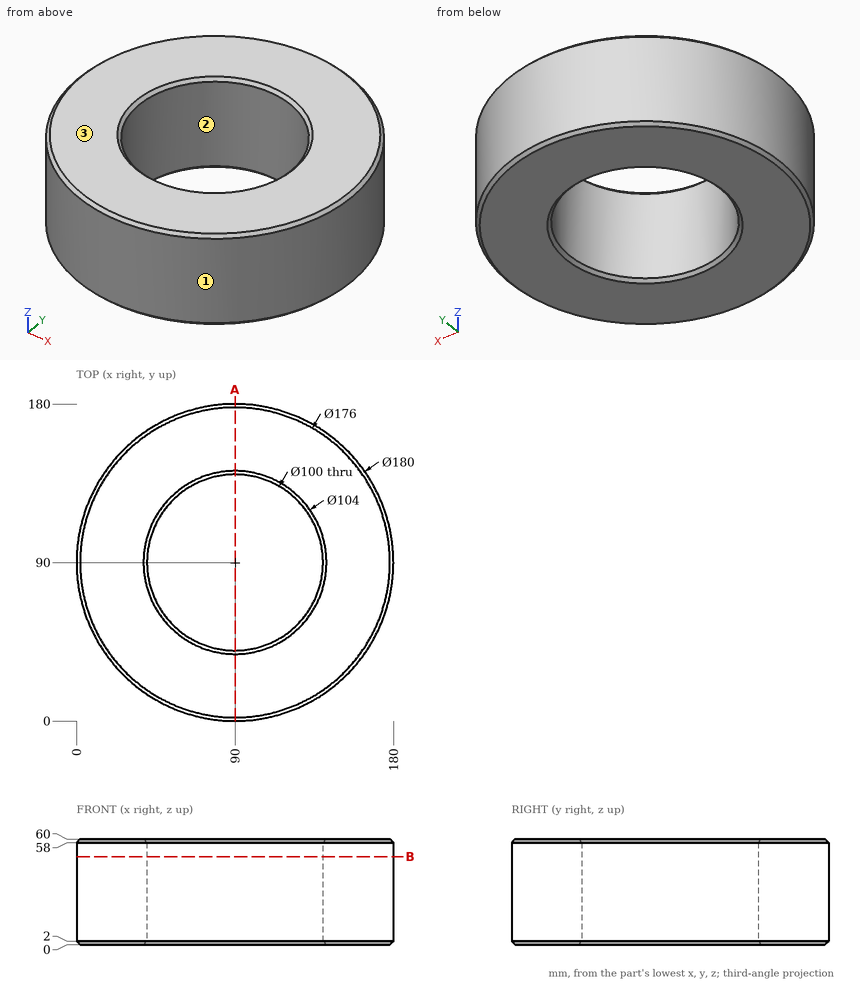
Here's the drawing with two shaded views (mm, measured from the low corner). I have some questions. Coordinates: 2 decimals unless noted, no trailing zeros. Write each loop counter-clockwise with the first axis right and the second up, starting at its lowest first coordinate (ties: lowest second). Pieces come first, ordered by that corner, then holes. Notation, with made-up numbers: M 43.25,37 L 80.25,37 A29 ccw 80.25,76 Z; hole C 6.5,77 d3. An arc over 180 degrees is marked long. Write item = value, one per line. Start each with the question number.
Q1. If we section it at B-B, the plane z = 50: Write out the boundary of the cut face in (x, y), then the cut area to 3 significant figures.
Q2. If I drill on L1, parallel to Y at x = 90, z = 33; L2, parallel to X at y = 95, z = 26; L3, parallel to X at y = 56.5, z = 24.5, over which ranges is the centre line in solid material (lowest first)? Write a range as [from, to].
Q3. I'm going to push flat-ended pins straight in: pin 1 (1 mm diameter, centred on y = 152, z = 47.5, fed in from +X); pin 2 (1 mm diameter, centred on y = 24.5, z = 40, fed in from -X); pin 3 (3 mm diameter, centred on x = 40, z = 44, fed in from +Y). Where does each tip first touch, or does it pass through?
Q4. Thinking about a two-plate mould opening in Y: for the marked faces 1, 2 and 3, which applies, released by +Y, released by -Y, zero draft, split by the parting line, or undercut?
Q5. If we section it at A-A, the plane x = 90: Write out the boundary of the cut face in (y, z).
Check sheet entries:
q1.outline = C 90,90 d180; hole C 90,90 d100
q1.area = 17,600 mm²
q2.L1 = [0, 40], [140, 180]
q2.L2 = [0.14, 40.25], [139.75, 179.86]
q2.L3 = [6.47, 52.88], [127.12, 173.53]
q3.pin_1 = 155.71
q3.pin_2 = 27.75
q3.pin_3 = 165.81
q4.face_1 = split by the parting line
q4.face_2 = undercut
q4.face_3 = zero draft
q5.outline = M 0,2 L 2,0 L 38,0 L 40,2 L 40,58 L 38,60 L 2,60 L 0,58 Z; M 140,2 L 142,0 L 178,0 L 180,2 L 180,58 L 178,60 L 142,60 L 140,58 Z
